```python
from build123d import *

# Parameters (mm, degrees)
SKETCH1_R           = 4
BOSS_EXTRUDE1_DEPTH = 1
SKETCH2_R           = 3.75
BOSS_EXTRUDE2_DEPTH = 1
SKETCH3_R           = 4
BOSS_EXTRUDE3_DEPTH = 6
SKETCH4_R           = 5
BOSS_EXTRUDE4_DEPTH = 2
CHAMFER1_SIZE       = 0.5


with BuildPart() as part:
    # Sketch1 → Boss-Extrude1 (new body)
    with BuildSketch(Plane.XY):
        Circle(SKETCH1_R)
    extrude(amount=BOSS_EXTRUDE1_DEPTH)

    # Sketch2 → Boss-Extrude2 (add)
    with BuildSketch(Plane.XY.offset(1)):
        Circle(SKETCH2_R)
    extrude(amount=BOSS_EXTRUDE2_DEPTH)

    # Sketch3 → Boss-Extrude3 (add)
    with BuildSketch(Plane.XY.offset(2)):
        Circle(SKETCH3_R)
    extrude(amount=BOSS_EXTRUDE3_DEPTH)

    # Sketch4 → Boss-Extrude4 (add)
    with BuildSketch(Plane.XY.offset(8)):
        Circle(SKETCH4_R)
    extrude(amount=BOSS_EXTRUDE4_DEPTH)

    # Chamfer1
    chamfer1_edges = [part.edges().sort_by_distance(p)[0] for p in [
        (-5, 0, 8),
        (-5, 0, 10),
        (-4, 0, 0),
    ]]
    chamfer(chamfer1_edges, length=CHAMFER1_SIZE)


solid = part.part
```
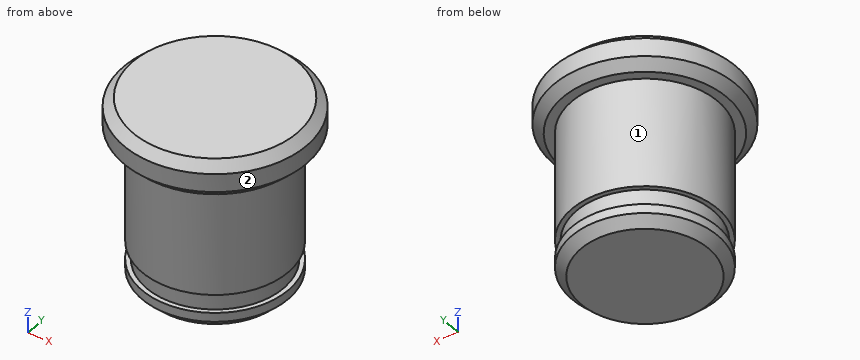
Design review of the part built by this model. Coordinates are the model's own, in mm. Face numbers are marked on the shaded views. A direction names the side the tool comes from. Give positions to 0.01 mm unless a question says otherwise; leave off trailing zeros. Loops run counter-clockwise (first coordinate to the right, second up) from the corner with the lowest first, then second, coordinate; pieces in that order, holes last. Notation, with made-up numbers: M -4,58 L 3,58 A13 ccw 3,83 Z; hole C 54.25,71.5 d4. An arc over 180 degrees is marked long. Return JSON: item names as keys, results as strings. Group by question number.
Item 1: Tool access review of the marked faces 1 and 2: name each direction out of +Z, -Z, +X, -X, +Y, -Y from which nothing blocks a thin tool from reaching the whole face with its end or side.
Item 2: For probe 1 along Z at (x, y) = (1.5, -3.5); probe 2 along Z at (x, y) = (3, 3.25); probe 3 along Z at (x, y) = (-2.5, -3), list the stretches that pass through material, from the lowest coordinate up.
Item 3: We need section C-C (z = 7.5). Give the boundary of the cut face in (x, y).
Item 4: We need section A-A (x = 0). Give the boundary of the cut face in (y, z).
Item 5: Insertion check: pin 1 Ø1.5 at (y, z) = (2.5, 4) entering from +X; pin 2 Ø2 at (y, z) = (-2, 8.5) entering from -X; pin 3 Ø3 at (y, z) = (1.5, 5.5) entering from +X. Each pin has a flat end and moves straight along its axis. Give the tip position at first contact, or say it passes through.
Output:
{
 "1": {"face 1": "-Z", "face 2": "+Z, -Z"},
 "2": {"probe 1": "z = 0.31 to 1, 2 to 10", "probe 2": "z = 8 to 10", "probe 3": "z = 0.41 to 1, 2 to 10"},
 "3": {"outline": "C 0,0 d8"},
 "4": {"outline": "M -5,8.5 L -4.5,8 L -4,8 L -4,2 L -3.75,2 L -3.75,1 L -4,1 L -4,0.5 L -3.5,0 L 3.5,0 L 4,0.5 L 4,1 L 3.75,1 L 3.75,2 L 4,2 L 4,8 L 4.5,8 L 5,8.5 L 5,9.5 L 4.5,10 L -4.5,10 L -5,9.5 Z"},
 "5": {"pin 1": "stops at x = 3.6", "pin 2": "stops at x = -4.9", "pin 3": "stops at x = 4"}
}
